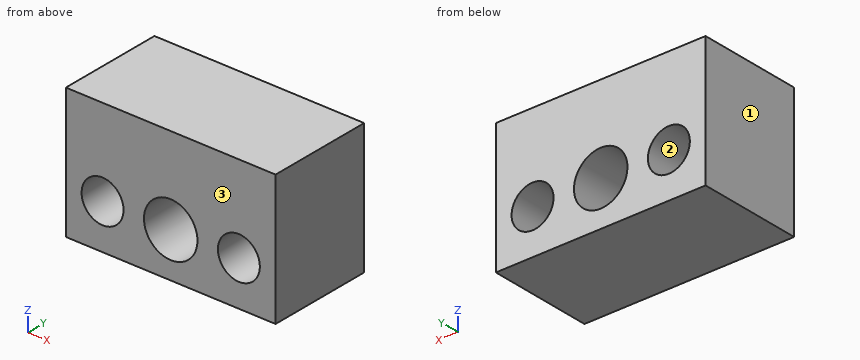
```python
from build123d import *

# Parameters (mm, degrees)
SKETCH_1_W              = 40
SKETCH_1_H              = 20
EXTRUDE_1_DEPTH         = 8.5
CUT_EXTRUDE_1_REACH     = 31.534
SKETCH_2_R              = 4
CUT_EXTRUDE_2_REACH     = 31.534
SKETCH_3_R              = 4
SKETCH_6_W              = 40
SKETCH_6_H              = 20
EXTRUDE_3_DEPTH         = 8
HOLE_WIZARD_M12_1_D     = 10.2
HOLE_WIZARD_M12_1_DEPTH = 20


with BuildPart() as part:
    # 草图1 → 凸台-拉伸1 (new, symmetric)
    with BuildSketch(Plane.XY):
        Rectangle(SKETCH_1_W, SKETCH_1_H)
    extrude(amount=EXTRUDE_1_DEPTH, both=True)

    # 草图2 → 切除-拉伸1 (cut, up to next)
    with BuildSketch(Plane(origin=(0, 10, 0), x_dir=(1, 0, 0), z_dir=(0, 1, 0)), mode=Mode.PRIVATE) as cut_extrude_1_sk1:
        with Locations(Location((-13, 0, 0), (0, 0, 270))):
            Circle(SKETCH_2_R)
    cut_extrude_1_tool1 = extrude(cut_extrude_1_sk1.sketch, amount=-CUT_EXTRUDE_1_REACH, mode=Mode.PRIVATE) & part.part
    # 草图2 → 切除-拉伸1 (cut, up to next)
    with BuildSketch(Plane(origin=(0, 10, 0), x_dir=(1, 0, 0), z_dir=(0, 1, 0)), mode=Mode.PRIVATE) as cut_extrude_1_sk2:
        with Locations(Location((13, 0, 0), (0, 0, 270))):
            Circle(SKETCH_2_R)
    cut_extrude_1_tool2 = extrude(cut_extrude_1_sk2.sketch, amount=-CUT_EXTRUDE_1_REACH, mode=Mode.PRIVATE) & part.part
    add(cut_extrude_1_tool1.solids().sort_by_distance((-13, 10, 0))[0], mode=Mode.SUBTRACT)
    add(cut_extrude_1_tool2.solids().sort_by_distance((13, 10, 0))[0], mode=Mode.SUBTRACT)

    # 草图3 → 切除-拉伸2 (cut, up to next)
    with BuildSketch(Plane.XZ.offset(10), mode=Mode.PRIVATE) as cut_extrude_2_sk1:
        with Locations(Location((0, 0, 0), (0, 0, 270))):
            Circle(SKETCH_3_R)
    cut_extrude_2_tool1 = extrude(cut_extrude_2_sk1.sketch, amount=-CUT_EXTRUDE_2_REACH, mode=Mode.PRIVATE) & part.part
    add(cut_extrude_2_tool1.solids().sort_by_distance((0, -10, 0))[0], mode=Mode.SUBTRACT)

    # 草图6 → 凸台-拉伸3 (add)
    with BuildSketch(Plane.XY.offset(8.5)):
        Rectangle(SKETCH_6_W, SKETCH_6_H)
    extrude(amount=EXTRUDE_3_DEPTH)

    # M12 螺纹孔1
    with Locations(Plane.ZX.offset(10)):
        with Locations((0, 0)):
            Hole(HOLE_WIZARD_M12_1_D / 2, depth=HOLE_WIZARD_M12_1_DEPTH)


solid = part.part
```
Geometry check sheet. Reference: the model listing, model coordinates, mm. Face numbers are marked on the shaded views. Give positions to 0.01 mm unless a question says otherwise; leave off trailing zeros. Loops run counter-clockwise (first coordinate to the right, second up) from the corner with the lowest first, then second, coordinate; pieces in that order, holes last. Notation, with made-up numbers: M 14,32 L 23,32 A23 ccw 23,59 Z; hole C -33.5,29 d4. An arc over 180 degrees is marked long. Write item = value, one per line. Start each with the question number.
1. Section check D-D, the plane x = 0. Enter the section's corners in (y, z).
2. Thickness scan on probe 1 along X at (y, z) = (-2.75, 0); probe 2 along X at (y, z) = (-3, 3.25); probe 3 along Z at (x, y) = (2, -7.75). Record the ranges inside material, lowest first.
3. Section check C-C, the plane z = 0. Enter the section's corners in (x, y), plus the area to 3 significant figures.
4. Section check A-A, the plane x = -13. Enter the section's corners in (y, z).
5. Draft check along X on the marked faces 1, 2 and 3. Enter one of: +X half, -X half, draft (parallel to the pull), parting line (faces both ways), or undercut.
6. Section check B-B, the plane y = 4. Enter the section's corners in (x, z), plus the area to 3 significant figures.
Values follow:
q1.outline = M -10,-8.5 L 10,-8.5 L 10,-5.1 L -10,-5.1 Z; M -10,5.1 L 10,5.1 L 10,16.5 L -10,16.5 Z
q2.probe_1 = -20 to -17, -9 to -5.1, 5.1 to 9, 17 to 20
q2.probe_2 = -20 to -15.33, -10.67 to -3.93, 3.93 to 10.67, 15.33 to 20
q2.probe_3 = -8.5 to -4.69, 4.69 to 16.5
q3.outline = M -20,-10 L -17,-10 L -17,10 L -20,10 Z; M -9,-10 L -5.1,-10 L -5.1,10 L -9,10 Z; M 5.1,-10 L 9,-10 L 9,10 L 5.1,10 Z; M 17,-10 L 20,-10 L 20,10 L 17,10 Z
q3.area = 276 mm^2
q4.outline = M -10,-8.5 L 10,-8.5 L 10,-4 L -10,-4 Z; M -10,4 L 10,4 L 10,16.5 L -10,16.5 Z
q5.face_1 = -X half
q5.face_2 = undercut
q5.face_3 = draft
q6.outline = M -20,-8.5 L 20,-8.5 L 20,16.5 L -20,16.5 Z; hole C -13,0 d8; hole C 0,0 d10.2; hole C 13,0 d8
q6.area = 818 mm^2
